from build123d import *

# Parameters (mm, degrees)
SKETCH1_W                  = 360
SKETCH1_H                  = 324
BOSS_EXTRUDE1_DEPTH        = 10
CHAMFER1_SIZE              = 25
FILLET1_R                  = 20
F_25_0_25_DIAMETER_HOLE1_D = 26


with BuildPart() as part:
    # Sketch1 → Boss-Extrude1 (new, symmetric)
    with BuildSketch(Plane.XY):
        with Locations((180, 162)):
            Rectangle(SKETCH1_W, SKETCH1_H)
    extrude(amount=BOSS_EXTRUDE1_DEPTH, both=True)

    # Chamfer1
    chamfer1_edges = [part.edges().sort_by_distance(p)[0] for p in [
        (0, 324, 0),
    ]]
    chamfer(chamfer1_edges, length=CHAMFER1_SIZE)

    # Fillet1
    fillet1_edges = [part.edges().sort_by_distance(p)[0] for p in [
        (360, 0, 0),
    ]]
    fillet(fillet1_edges, radius=FILLET1_R)

    # Ø25.0 (25) Diameter Hole1 (through all)
    with Locations(Plane.XY.offset(10)):
        with Locations((85, 33), (325, 33), (325, 273), (85, 273)):
            Hole(F_25_0_25_DIAMETER_HOLE1_D / 2)


solid = part.part
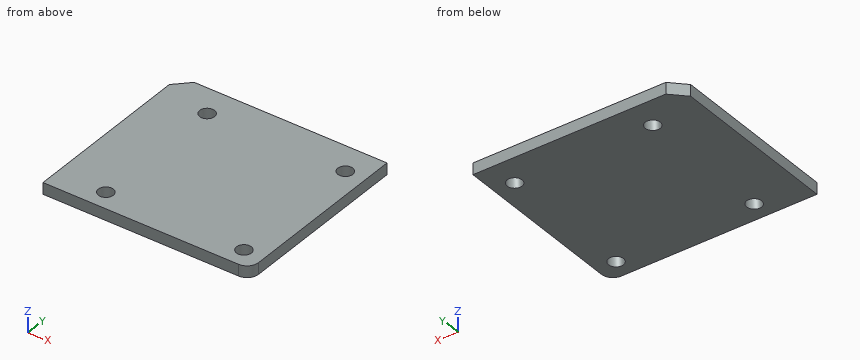
Check sheet for the modelled part. Datum: model origin and axes. Units: mm. Round coordinates to 2 decimals unless told otherwise and drop trailing zeros. Write each loop counter-clockwise with the first axis right and the second up, starting at its lowest first coordinate (ties: lowest second). Pieces come first, ordered by that corner, then holes. Notation, with made-up numbers: (-14.5, -29.75) -> (-5.5, -29.75) arc R22 cw to (-5.5, -14.75) -> close; hole circle Ø10 at (4, 87.5). An arc over 180 degrees is marked (long way). Answer as CSV lines item,"result". Start each with the question number.
1) Section check C-C on z = -3.75. Enter the section's corners in (x, y), and give its area (3 significant figures).
2) Section check B-B on x = 325. Enter the section's corners in (y, z).
3) Go/stop test with a flat-tipped pin: P1, Ø23.5, axis at x = 325, y = 273, coming from the +Z side. Record where the tip stops, or that it passes through.
4) Material ranges on line 1 (Y direction, x = 325, z = 0.75); line 2 (X direction, y = 275, z = -2.5); line 3 (X direction, y = 41, z = -4.25), recorded low to high. Write a range as from..to.
5) Section check A-A on y = 273. Enter the section's corners in (x, z), and give its area (3 significant figures).
Found:
1,outline,"(0, 0) -> (340, 0) arc R20 ccw to (360, 20) -> (360, 324) -> (25, 324) -> (0, 299) -> close; hole circle Ø26 at (85, 33); hole circle Ø26 at (85, 273); hole circle Ø26 at (325, 33); hole circle Ø26 at (325, 273)"
1,area,"114,000 mm^2"
2,outline,"(0, -10) -> (20, -10) -> (20, 10) -> (0, 10) -> close; (46, -10) -> (260, -10) -> (260, 10) -> (46, 10) -> close; (286, -10) -> (324, -10) -> (324, 10) -> (286, 10) -> close"
3,P1,"passes through"
4,line 1,"y = 0..20, 46..260, 286..324"
4,line 2,"x = 0..72.15, 97.85..312.15, 337.85..360"
4,line 3,"x = 0..74.75, 95.25..314.75, 335.25..360"
5,outline,"(0, -10) -> (72, -10) -> (72, 10) -> (0, 10) -> close; (98, -10) -> (312, -10) -> (312, 10) -> (98, 10) -> close; (338, -10) -> (360, -10) -> (360, 10) -> (338, 10) -> close"
5,area,"6,160 mm^2"
